Can you work these out from the model? Positions are in its coordinate system, mm. Coordinates: 2 decimals unless noted, no trailing zeros. Write each loop counter-clockwise with the first axis right and the second up, starting at its lowest first coordinate (ties: lowest second). Pieces come first, ordered by that corner, then holes. Notation, with made-up numbers: (-37.75, -5) - (-13.75, -5) arc R19 ccw to (-13.75, 13) - close; hole circle Ø10 at (84, -0.5). An arc over 180 degrees is marked (long way). Use one line per item in the form item = value. Start each with the question number.
(1) For pin 1 Ø0.9 at (x, z) = (58, 1) entering from +Y; pin 2 Ø3.5 at (x, y) = (0, 33.25) entering from +Z, each with a flat end and sliding along its axis, tell me the tip position at first contact or that it passes through.
(2) If we section it at D-D on y = -16: Please give me the cut outline in (x, z).
(3) If we section it at C-C on x = -33.25: Please give me the cut outline in (y, z), then the cut area to 3 significant figures.
(4) Thinking about a two-plate mould opening in Y: for faces 1 (the face through (-21.3, 1.3, 3)), 2 (the face through (-0.52, -18.33, 0.34)), 3 (the face through (41.53, -79.845, 1.479)), which applies, pulls with the +Y half, pulls with the -Y half, needs draft (parallel to the pull), parting line crosses it, or undercut?
(5) If we section it at A-A on z = 2.1: Give the number of separate pieces and of enclosed holes in the cut face, then the cut area to 3 significant figures.
(6) If we section it at B-B on x = 0: Please give me the cut outline in (y, z).
(7) If I drill on probe 1 along Y at (x, z) = (0, 0.9); probe 2 along Y at (x, z) = (32.5, 2.7); probe 3 along X at (y, z) = (-16, 2.4), over which ranges is the centre line in solid material (lowest first)? Write a range as from..to.
```python
from build123d import *

# Parameters (mm, degrees)
SKETCH1_R           = 90
SKETCH1_R_2         = 10
BOSS_EXTRUDE1_DEPTH = 3
SKETCH2_R           = 2.25
SKETCH2_R_2         = 2.75
CUT_EXTRUDE1_DEPTH  = 3
CHAMFER1_SIZE       = 2.8


with BuildPart() as part:
    # Sketch1 → Boss-Extrude1 (new body)
    with BuildSketch(Plane.XY):
        Circle(SKETCH1_R)
        Circle(SKETCH1_R_2, mode=Mode.SUBTRACT)
    extrude(amount=BOSS_EXTRUDE1_DEPTH)

    # Sketch2 → Cut-Extrude1 (cut)
    with BuildSketch(Plane.XY.offset(3)):
        with Locations((0, 16)):
            Circle(SKETCH2_R)
        with Locations((-16, 0)):
            Circle(SKETCH2_R)
        with Locations((0, -16)):
            Circle(SKETCH2_R)
        with Locations((16, 0)):
            Circle(SKETCH2_R)
        with Locations((0, 33.25)):
            Circle(SKETCH2_R_2)
        with Locations((-33.25, 0)):
            Circle(SKETCH2_R_2)
        with Locations((0, -33.25)):
            Circle(SKETCH2_R_2)
        with Locations((33.25, 0)):
            Circle(SKETCH2_R_2)
        with BuildLine():
            Line((50, 3.1), (75, 3.1))
            ThreePointArc((75, 3.1), (78.1, 0), (75, -3.1))
            Line((75, -3.1), (50, -3.1))
            ThreePointArc((50, -3.1), (46.9, 0), (50, 3.1))
        make_face()
    extrude(amount=-CUT_EXTRUDE1_DEPTH, mode=Mode.SUBTRACT)

    # Chamfer1
    chamfer1_edges = [part.edges().sort_by_distance(p)[0] for p in [
        (-2.25, 16, 3),
        (-18.25, 0, 3),
        (-2.25, -16, 3),
        (13.75, 0, 3),
    ]]
    chamfer(chamfer1_edges, length=CHAMFER1_SIZE)


solid = part.part
```
Reported:
q1.pin_1 = 69.2
q1.pin_2 = through
q2.outline = (-88.57, 0) - (-2.25, 0) - (-2.25, 0.2) - (-5.05, 3) - (-88.57, 3) - close; (2.25, 0) - (88.57, 0) - (88.57, 3) - (5.05, 3) - (2.25, 0.2) - close
q3.outline = (-83.63, 0) - (-2.75, 0) - (-2.75, 3) - (-83.63, 3) - close; (2.75, 0) - (83.63, 0) - (83.63, 3) - (2.75, 3) - close
q3.area = 485 mm2
q4.face_1 = needs draft
q4.face_2 = undercut
q4.face_3 = parting line crosses it
q5.separate_pieces = 1
q5.enclosed_holes = 10
q5.area = 24,600 mm2
q6.outline = (-90, 0) - (-36, 0) - (-36, 3) - (-90, 3) - close; (-30.5, 0) - (-18.25, 0) - (-18.25, 0.2) - (-21.05, 3) - (-30.5, 3) - close; (-13.75, 0) - (-10, 0) - (-10, 3) - (-10.95, 3) - (-13.75, 0.2) - close; (10, 0) - (13.75, 0) - (13.75, 0.2) - (10.95, 3) - (10, 3) - close; (18.25, 0) - (30.5, 0) - (30.5, 3) - (21.05, 3) - (18.25, 0.2) - close; (36, 0) - (90, 0) - (90, 3) - (36, 3) - close
q7.probe_1 = -90..-36, -30.5..-18.95, -13.05..-10, 10..13.05, 18.95..30.5, 36..90
q7.probe_2 = -83.93..-2.65, 2.65..83.93
q7.probe_3 = -88.57..-4.45, 4.45..88.57
